For this review, use the dimensioned drawing (mm, ordinates from the lowest corner) and the shaded views. Give positions to 0.01 mm unless a question says otherwise; leave off trailing zeros. Write each loop counter-clockwise with the first axis right and the second up, starting at its lowest first coordinate (ties: lowest second). Pieces come first, ordered by that corner, then holes. Notation, with made-up numbers: (-13.5, 70) -> (4.5, 70) arc R22 cw to (4.5, 90) -> close; hole circle Ø6 at (28.5, 12). An arc over 180 degrees is marked (long way). Return JSON: item names as keys, results as strings.
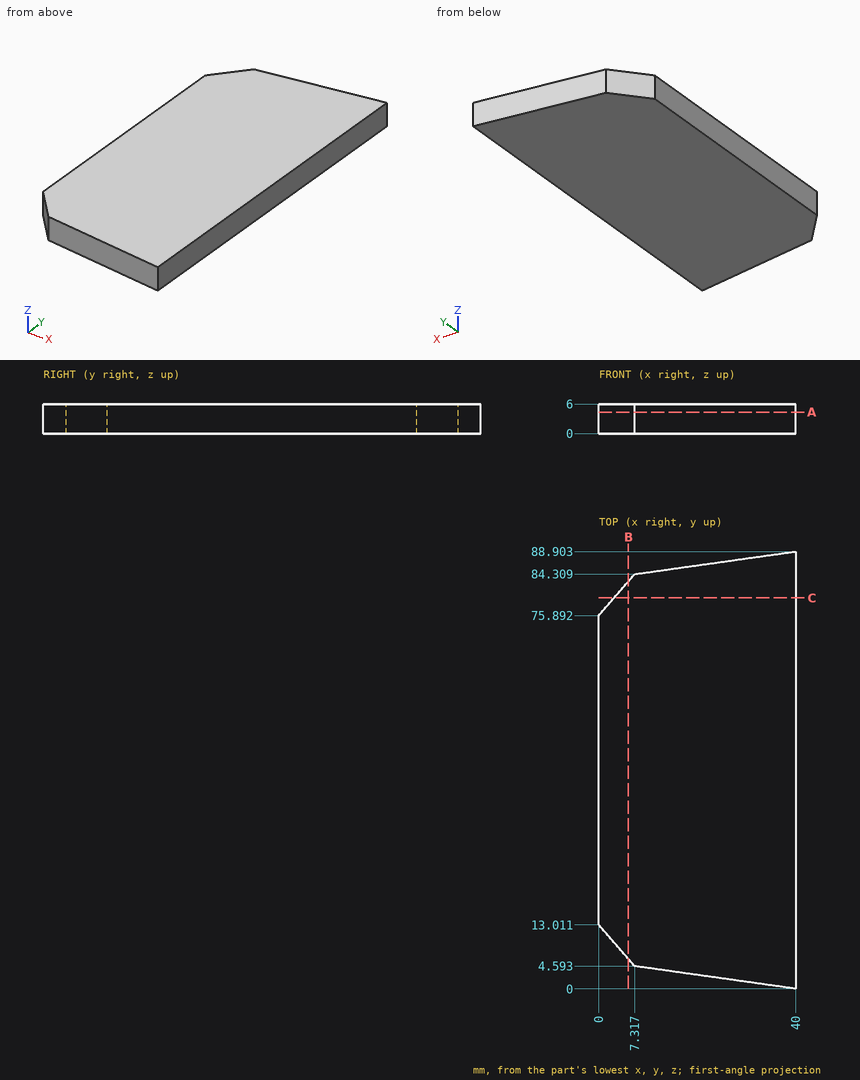
1. To check wall thickness, follow probe 1 along Y at (x, z) = (37, 4.45); probe 2 along Y at (x, z) = (10, 3); probe 3 along X at (y, z) = (12, 2.75). State the ranges of each line that lie inside material, in increasing order.
Results found:
{"probe 1": "y = 0.42 to 88.48", "probe 2": "y = 4.22 to 84.69", "probe 3": "x = 0.88 to 40"}
2. For pin 1 (1.5 mm diameter, centred on x = 9.5, z = 2.5, fed in from +Y); pin 2 (1.5 mm diameter, centred on x = 20, z = 3, fed in from +Y), all flat-tipped, find the tip position at first contact; note any pin that passes through.
Results found:
{"pin 1": "stops at y = 84.72", "pin 2": "stops at y = 86.2"}
3. Add section B-B, the plane x = 6. State the section outline as (y, z) points (1 decimal).
Results found:
{"outline": "(6.1, 0) -> (82.8, 0) -> (82.8, 6) -> (6.1, 6) -> close"}
4. Add section A-A, the plane z = 4.35. State the section outline as (x, y) points, plus the area to 3 significant figures.
Results found:
{"outline": "(0, 13.01) -> (7.32, 4.59) -> (40, 0) -> (40, 88.9) -> (7.32, 84.31) -> (0, 75.89) -> close", "area": "3,280 mm²"}
5. Add section C-C, the plane y = 79.5. State the section outline as (x, z) points, plus the area to 3 significant figures.
Results found:
{"outline": "(3.14, 0) -> (40, 0) -> (40, 6) -> (3.14, 6) -> close", "area": "221 mm²"}
